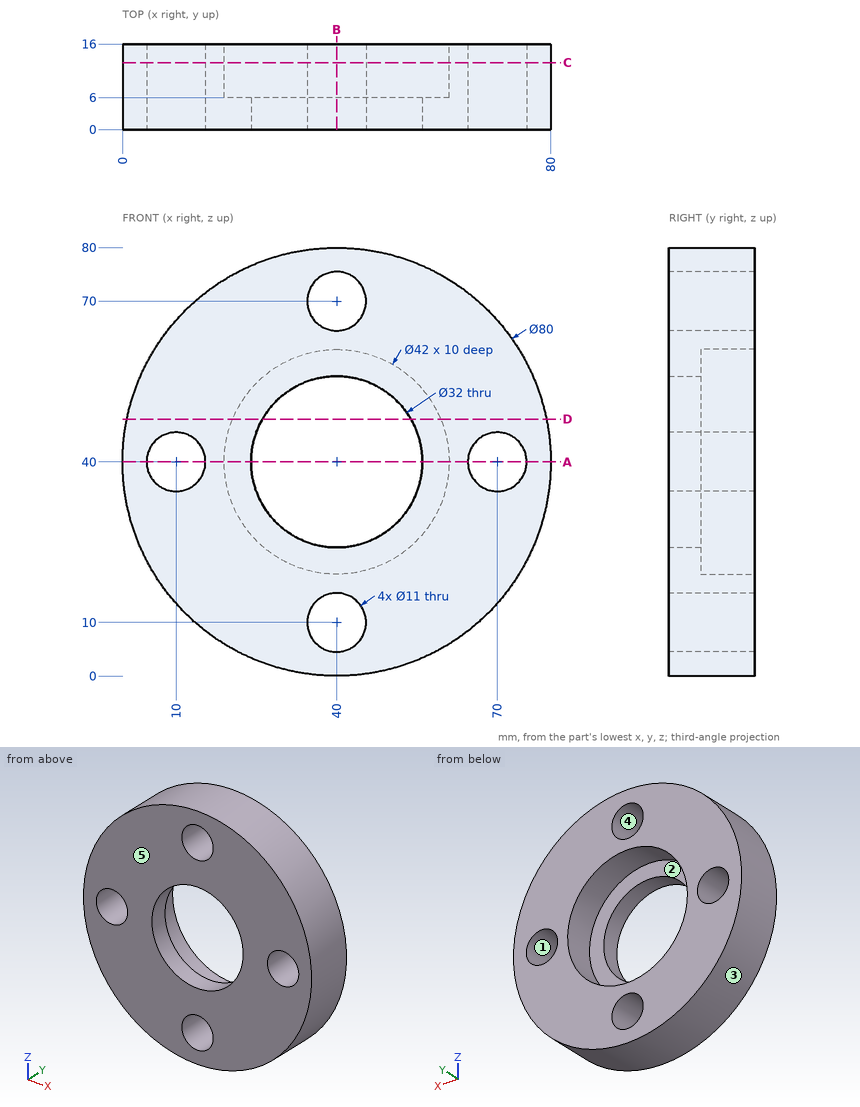
Here's the drawing with two shaded views (mm, measured from the low corner). I have some questions. A direction names the side the tool comes from. Give positions to 0.01 mm unless a question says otherwise; leave off trailing zeros. Loops run counter-clockwise (first coordinate to the right, second up) from the corner with the lowest first, then second, coordinate; pieces in that order, holes last. Notation, with made-up numbers: (34.25, 68.25) -> (88.25, 68.25) arc R19 ccw to (88.25, 102.25) -> close; hole circle Ø10 at (44.25, 47.25). An arc over 180 degrees is marked (long way). Use one line per item in the form item = value.
1) If we section it at A-A (z = 40): Please give me the cut outline in (x, y), plus the area to 3 significant figures.
Answers:
outline = (0, 0) -> (4.5, 0) -> (4.5, 16) -> (0, 16) -> close; (15.5, 0) -> (24, 0) -> (24, 6) -> (19, 6) -> (19, 16) -> (15.5, 16) -> close; (56, 0) -> (64.5, 0) -> (64.5, 16) -> (61, 16) -> (61, 6) -> (56, 6) -> close; (75.5, 0) -> (80, 0) -> (80, 16) -> (75.5, 16) -> close
area = 316 mm²
2) If we section it at C-C (y = 12.5): Please give me the cut outline in (x, z), plus the area to 3 significant figures.
Answers:
outline = circle Ø80 at (40, 40); hole circle Ø11 at (10, 40); hole circle Ø42 at (40, 40); hole circle Ø11 at (40, 10); hole circle Ø11 at (40, 70); hole circle Ø11 at (70, 40)
area = 3,260 mm²
3) For the marked faces 1 and 2, which set-ups out of +Z, -Z, +X, -X, +Y, -Y let a thin tool reach every point of the face, with its end or its side?
Answers:
face_1 = +Y, -Y
face_2 = +Y
4) Will these pins go through, and if not, where does the flat tip stop? pin 1 (5 mm diameter, centred on x = 69, y = 10.5, fed in from -Z); pin 2 (1.5 mm diameter, centred on x = 39, y = 14.5, fed in from -Z); pin 3 (1.5 mm diameter, centred on x = 54, y = 11, fed in from -Z); pin 4 (10 mm diameter, centred on x = 40, z = 10, fed in from +Y).
Answers:
pin_1 = 10.04
pin_2 = 0
pin_3 = 2.26
pin_4 = through
5) If we section it at B-B (x = 40): Please give me the cut outline in (y, z).
Answers:
outline = (0, 0) -> (16, 0) -> (16, 4.5) -> (0, 4.5) -> close; (0, 15.5) -> (16, 15.5) -> (16, 19) -> (6, 19) -> (6, 24) -> (0, 24) -> close; (0, 56) -> (6, 56) -> (6, 61) -> (16, 61) -> (16, 64.5) -> (0, 64.5) -> close; (0, 75.5) -> (16, 75.5) -> (16, 80) -> (0, 80) -> close
6) We'd pull the mould along Z, two halves only. Please class the marked faces 3, 4 and 5: released by +Z, released by -Z, zero draft, split by the parting line, or undercut.
Answers:
face_3 = split by the parting line
face_4 = undercut
face_5 = zero draft
7) I need wall thicknesses on line 1 along X through (y, z) = (9, 40); line 2 along X through (y, z) = (8.25, 12.5); line 3 along X through (y, z) = (6.5, 70). Which ranges of each line are inside material? Lowest first, please.
Answers:
line_1 = 0 to 4.5, 15.5 to 19, 61 to 64.5, 75.5 to 80
line_2 = 10.95 to 35.1, 44.9 to 69.05
line_3 = 13.54 to 34.5, 45.5 to 66.46
8) If we section it at D-D (z = 48): Please give me the cut outline in (x, y).
Answers:
outline = (0.81, 0) -> (26.14, 0) -> (26.14, 6) -> (20.58, 6) -> (20.58, 16) -> (0.81, 16) -> close; (53.86, 0) -> (79.19, 0) -> (79.19, 16) -> (59.42, 16) -> (59.42, 6) -> (53.86, 6) -> close
